Check sheet for the drawn part. Datum: minimum x, y, z corner. Units: mm. A direction names the side the tool comes from. Round coordinates to 2 decimals unless told otherwise and drop trailing zeros. Loops run counter-clockwise (first coordinate to the right, second up) from the corner with the lowest first, then second, coordinate; pieces in that order, holes last.
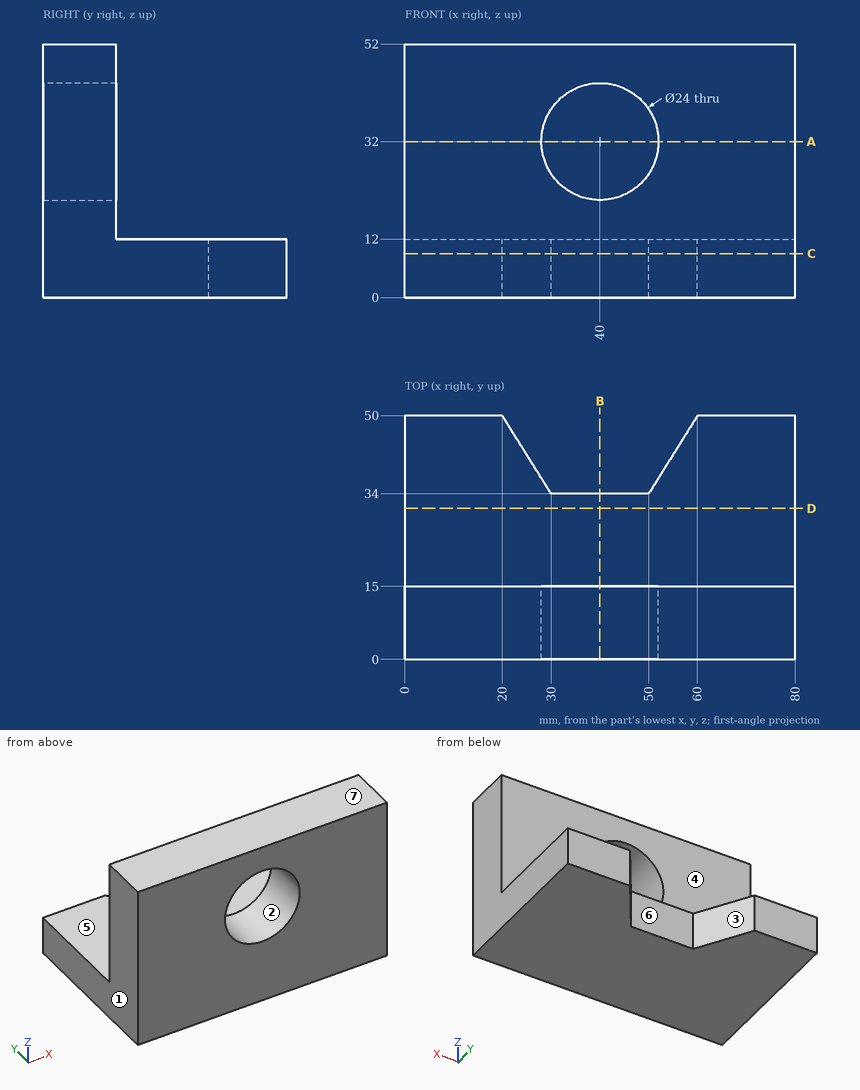
1) Scan lines: line 1 along X through (y, z) = (7, 32); line 2 along Z through (x, y) = (12.5, 31); line 3 along Y through (x, z) = (58.5, 12.5). Record each from-to range of solid material in increasing order.
Report:
line 1: x = 0 to 28, 52 to 80
line 2: z = 0 to 12
line 3: y = 0 to 15
2) Gauge pin test, flat ends, axial feed: pin 1 (12 mm diameter, centred on x = 22, z = 41.5, fed in from +Y); pin 2 (4 mm diameter, centred on x = 54, z = 44, fed in from -Y); pin 3 (3 mm diameter, centred on x = 43.5, y = 23, fed in from +Z); pin 4 (6 mm diameter, centred on x = 40, z = 5, fed in from +Y). Record the tip position at first contact, or that the pin passes through.
Report:
pin 1: stops at y = 15
pin 2: stops at y = 0
pin 3: stops at z = 12
pin 4: stops at y = 34
3) Sectioned sample at D-D, the plane y = 31. Record the cut outline in (x, z), then the cut area to 3 significant figures.
Report:
outline: (0, 0) - (80, 0) - (80, 12) - (0, 12) - close
area: 960 mm2
4) Sectioned sample at B-B, the plane x = 40. Record the cut outline in (y, z), then the cut area to 3 significant figures.
Report:
outline: (0, 0) - (34, 0) - (34, 12) - (15, 12) - (15, 20) - (0, 20) - close; (0, 44) - (15, 44) - (15, 52) - (0, 52) - close
area: 648 mm2
5) Sectioned sample at A-A, the plane z = 32. Record the cut outline in (x, y).
Report:
outline: (0, 0) - (28, 0) - (28, 15) - (0, 15) - close; (52, 0) - (80, 0) - (80, 15) - (52, 15) - close
6) Mould release check, pull along X, two halves, no side actions. Record for the marked faces 1, 2, 3 and 4: +X half, -X half, draft (parallel to the pull), parting line (faces both ways), or undercut.
Report:
face 1: -X half
face 2: undercut
face 3: undercut
face 4: draft
7) Access from +Z, -Z, +X, -X, +Y, -Y to the whole of each face (thin tool, end or side, straight path). Record for the marked faces 5, 6 and 7.
Report:
face 5: +Z, +X, -X, +Y
face 6: +Z, -Z, +Y
face 7: +Z, +X, -X, +Y, -Y
8) Sectioned sample at C-C, the plane z = 9. Record the cut outline in (x, y).
Report:
outline: (0, 0) - (80, 0) - (80, 50) - (60, 50) - (50, 34) - (30, 34) - (20, 50) - (0, 50) - close
